Model file for the job. Use its own axes, mm. Face numbers are marked on the shaded views. A direction names the side the tool comes from. Coordinates: 2 decimals unless noted, no trailing zeros. Order: outer loops, then holes, each group sorted by start corner. A loop starts at its lowest first (then second) coordinate and runs counter-clockwise, first axis right, second up. Notation, with made-up numbers: (12, 25) -> (39, 25) arc R6 cw to (39, 35) -> close; hole circle Ø3 at (54.5, -1). An arc over 180 degrees is marked (long way). Write item = value, one per line. Start each with the question number.
Q1. Cut at C-C, the plane y = -14.5. List the corners of the cut face in (x, z), plus the area to 3 significant figures.
Q2. Cut at A-A, the plane z = 11.5. List the corners of the cut face in (x, y), plus the area to 3 significant figures.
Q3. Cut at D-D, the plane z = 18. List the corners of the cut face in (x, y).
Q4. Flat gauge pins, fed straight in: pin 1 (1.5 mm diameter, centred on y = 17, z = 10.5, fed in from +X); pin 2 (6.5 mm diameter, centred on y = -36, z = 17, fed in from -X); pin 3 (3 mm diameter, centred on y = -33.5, z = 18.5, fed in from +X); pin 4 (5 mm diameter, centred on x = -24.5, y = -35.5, fed in from -Z). Where does each tip first touch, or does it go through?
Q5. Cut at B-B, the plane x = 39. List the corners of the cut face in (y, z), plus the area to 3 significant figures.
Q6. 3-axis set-ups, long thin cutter, end or side, ignore diameter. For the marked faces 4, 5 and 6: which of +Z, -Z, +X, -X, +Y, -Y reach the whole face in a straight line?
Q7. Mould opens along Y. For the marked faces 1, 2 and 3 say: +Y half, -Y half, draft (parallel to the pull), parting line (faces both ways), or undercut.
Q8. Wall check: line 1 (Y direction, x = 17.5, z = 17.75); line 2 (Y direction, x = 38.5, z = 2.25); line 3 (Z direction, x = -23, y = -13.5). Give the ranges that are in metal, low to high. Write a range as from..to.
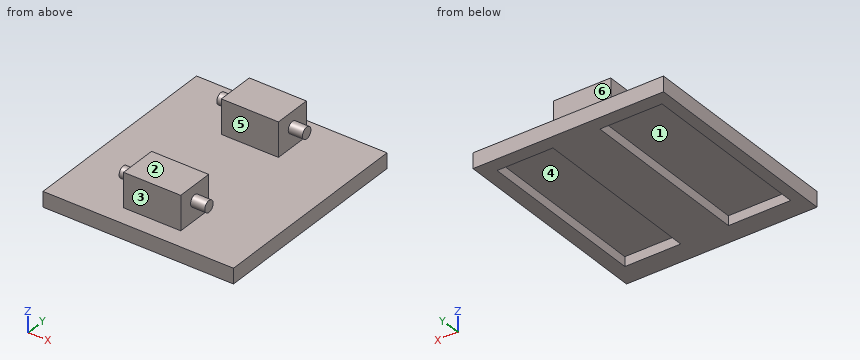
from build123d import *

# Parameters (mm, degrees)
SKETCH1_W           = 100
SKETCH1_H           = 110
BOSS_EXTRUDE1_DEPTH = 8
SKETCH2_W           = 30
SKETCH2_H           = 20
BOSS_EXTRUDE2_DEPTH = 18
SKETCH4_W           = 29.345369705
SKETCH4_H           = 91.568125834
SKETCH4_W_2         = 32.679168461
SKETCH4_H_2         = 92.103849907
CUT_EXTRUDE2_DEPTH  = 5
SKETCH3_R           = 3
BOSS_EXTRUDE3_DEPTH = 22.5


with BuildPart() as part:
    # Sketch1 → Boss-Extrude1 (new body)
    with BuildSketch(Plane.XY):
        Rectangle(SKETCH1_W, SKETCH1_H)
    extrude(amount=BOSS_EXTRUDE1_DEPTH)

    # Sketch2 → Boss-Extrude2 (add)
    with BuildSketch(Plane.XY.offset(8)):
        with Locations((0, 35)):
            Rectangle(SKETCH2_W, SKETCH2_H)
        with Locations((0, -35)):
            Rectangle(SKETCH2_W, SKETCH2_H)
    extrude(amount=BOSS_EXTRUDE2_DEPTH)

    # Sketch4 → Cut-Extrude2 (cut)
    with BuildSketch(Plane(origin=(0, 0, 0), x_dir=(-1, 0, 0), z_dir=(0, 0, -1))):
        with Locations((-27.976499336, 2.033263611)):
            Rectangle(SKETCH4_W, SKETCH4_H)
        with Locations((27.679077111, 1.765401575)):
            Rectangle(SKETCH4_W_2, SKETCH4_H_2)
    extrude(amount=-CUT_EXTRUDE2_DEPTH, mode=Mode.SUBTRACT)

    # Sketch3 → Boss-Extrude3 (add, symmetric)
    with BuildSketch(Plane(origin=(0, 0, 0), x_dir=(0, 0, -1), z_dir=(1, 0, 0))):
        with Locations(Location((-18, 35, 0), (0, 0, 180))):
            Circle(SKETCH3_R)
        with Locations(Location((-18, -35, 0), (0, 0, 180))):
            Circle(SKETCH3_R)
    extrude(amount=BOSS_EXTRUDE3_DEPTH, both=True)


solid = part.part
Here are the results:
q1.outline = (-50, 0) -> (-44.02, 0) -> (-44.02, 5) -> (-11.34, 5) -> (-11.34, 0) -> (13.3, 0) -> (13.3, 5) -> (42.65, 5) -> (42.65, 0) -> (50, 0) -> (50, 8) -> (-50, 8) -> close
q1.area = 490 mm²
q2.outline = (-15, -45) -> (15, -45) -> (15, -25) -> (-15, -25) -> close; (-15, 25) -> (15, 25) -> (15, 45) -> (-15, 45) -> close
q2.area = 1,200 mm²
q3.outline = (-22.5, -38) -> (-15, -38) -> (-15, -45) -> (15, -45) -> (15, -38) -> (22.5, -38) -> (22.5, -32) -> (15, -32) -> (15, -25) -> (-15, -25) -> (-15, -32) -> (-22.5, -32) -> close; (-22.5, 32) -> (-15, 32) -> (-15, 25) -> (15, 25) -> (15, 32) -> (22.5, 32) -> (22.5, 38) -> (15, 38) -> (15, 45) -> (-15, 45) -> (-15, 38) -> (-22.5, 38) -> close
q4.pin_1 = through
q4.pin_2 = -22.5
q4.pin_3 = 22.5
q4.pin_4 = 5
q5.outline = (-55, 0) -> (-43.75, 0) -> (-43.75, 5) -> (47.82, 5) -> (47.82, 0) -> (55, 0) -> (55, 8) -> (-55, 8) -> close
q5.area = 422 mm²
q6.face_4 = -Z
q6.face_5 = +Z, +X, -X
q6.face_6 = +Z, +X, -X, +Y
q7.face_1 = undercut
q7.face_2 = draft
q7.face_3 = -Y half
q8.line_1 = -37.99..-32.01, 32.01..37.99
q8.line_2 = -55..-43.75, 47.82..55
q8.line_3 = 5..8
